For this review, take the finished solid that the model builds, in its own axes (mm). Face numbers are marked on the shaded views. A direction names the side the tool comes from. Give positions to 0.01 mm unless a question says otherwise; leave off trailing zeros. Write each loop counter-clockwise with the first axis right and the second up, starting at its lowest first coordinate (ties: lowest second). Pieces come first, ordered by that corner, then holes.
1) Machinability: for the marked faces 5, 6, 7 and 8, which of the approach directions +Z, -Z, +X, -X, +Y, -Y give a long, thin tool a straight path to every point of the face, cutting with its end or side? Answer none if there is none.
2) Draft analysis for pull direction Y (two halves, no side actions). For the marked faces 1, 2, 3 and 4, state which applies: pulls with the +Y half, pulls with the -Y half, needs draft (parallel to the pull), parting line crosses it, or undercut.
3) We need section C-C on z = -5. Give the boundary of the cut face in (x, y).
4) For P1, Ø3, axis at x = 12.5, z = 9.5, coming from the -Y side; P2, Ø2, axis at x = 26.5, y = -0.5, coming from the -Z side; P3, Ø2.5, axis at y = 6, z = 8.5, coming from the -X side; P4, Ø8.5, axis at x = 0, y = 0, coming from the +Z side, all flat-tipped, find the tip position at first contact; note any pin that passes through.
5) We need section B-B on z = 10. Give the boundary of the cut face in (x, y), and give its area (3 significant figures).
6) Wall thickness on line 1 along Y through (x, z) = (0, -7.25); line 2 along Z through (x, y) = (-16, -20); line 3 along Z through (x, y) = (18.5, -28.5): over which ranges is each line inside the solid? List them lowest first.
7) We need section A-A on x = 0. Give the boundary of the cut face in (y, z).
8) We need section D-D on y = -15. Give the boundary of the cut face in (x, z), and give its area (3 significant figures).
from build123d import *

# Parameters (mm, degrees)
BACK_DISC_SKETCH_R        = 37.5
BACK_DISC_75_DEPTH        = 3
BLADES_6X_DEPTH           = 14
HUB_SKETCH_R              = 12.5
HUB_25_DEPTH              = 16
KEYED_SHAFT_BORE_14_DEPTH = 63.461988441


with BuildPart() as part:
    # Back Disc Sketch → Back Disc Ø75 (new body)
    with BuildSketch(Plane.XY):
        Circle(BACK_DISC_SKETCH_R)
    extrude(amount=BACK_DISC_75_DEPTH)

    # Blade Profiles Sketch → Blades 6x (add)
    with BuildSketch(Plane.XY.offset(3)):
        with BuildLine():
            ThreePointArc((3.63084944, 16.288815705), (11.178007051, 25.36087614), (21.79252918, 30.51779271))
            Line((21.79252918, 30.51779271), (18.431665522, 32.657674536))
            ThreePointArc((18.431665522, 32.657674536), (8.308835539, 26.888544841), (1.030700016, 17.790012675))
            Line((1.030700016, 17.790012675), (3.63084944, 16.288815705))
        make_face()
        with BuildLine():
            ThreePointArc((-12.291103478, 11.288815705), (-16.374159474, 22.36087614), (-15.532919164, 34.131780238))
            Line((-15.532919164, 34.131780238), (-19.066543016, 32.291127844))
            ThreePointArc((-19.066543016, 32.291127844), (-19.131745134, 20.639935074), (-14.891252903, 9.787618735))
            Line((-14.891252903, 9.787618735), (-12.291103478, 11.288815705))
        make_face()
        with BuildLine():
            ThreePointArc((-15.921952918, -5), (-27.552166525, -3), (-37.325448345, 3.613987528))
            Line((-37.325448345, 3.613987528), (-37.498208538, -0.366546692))
            ThreePointArc((-37.498208538, -0.366546692), (-27.440580673, -6.248609768), (-15.921952918, -8.00239394))
            Line((-15.921952918, -8.00239394), (-15.921952918, -5))
        make_face()
        with BuildLine():
            ThreePointArc((-3.63084944, -16.288815705), (-11.178007051, -25.36087614), (-21.79252918, -30.51779271))
            Line((-21.79252918, -30.51779271), (-18.431665522, -32.657674536))
            ThreePointArc((-18.431665522, -32.657674536), (-8.308835539, -26.888544841), (-1.030700016, -17.790012675))
            Line((-1.030700016, -17.790012675), (-3.63084944, -16.288815705))
        make_face()
        with BuildLine():
            ThreePointArc((12.291103478, -11.288815705), (16.374159474, -22.36087614), (15.532919164, -34.131780238))
            Line((15.532919164, -34.131780238), (19.066543016, -32.291127844))
            ThreePointArc((19.066543016, -32.291127844), (19.131745134, -20.639935074), (14.891252903, -9.787618735))
            Line((14.891252903, -9.787618735), (12.291103478, -11.288815705))
        make_face()
        with BuildLine():
            ThreePointArc((15.921952918, 5), (27.552166525, 3), (37.325448345, -3.613987528))
            Line((37.325448345, -3.613987528), (37.498208538, 0.366546692))
            ThreePointArc((37.498208538, 0.366546692), (27.440580673, 6.248609768), (15.921952918, 8.00239394))
            Line((15.921952918, 8.00239394), (15.921952918, 5))
        make_face()
    extrude(amount=BLADES_6X_DEPTH)

    # Hub Sketch → Hub Ø25 (add)
    with BuildSketch(Plane(origin=(0, 0, 0), x_dir=(-1, 0, 0), z_dir=(0, 0, -1))):
        Circle(HUB_SKETCH_R)
    extrude(amount=HUB_25_DEPTH)

    # Shaft Bore Sketch → Keyed Shaft Bore Ø14 (cut, through all)
    with BuildSketch(Plane(origin=(0, 0, -16), x_dir=(-1, 0, 0), z_dir=(0, 0, -1))):
        with BuildLine():
            Line((-2.5, 6.538348415), (-2.5, 9.3))
            Line((-2.5, 9.3), (2.5, 9.3))
            Line((2.5, 9.3), (2.5, 6.538348415))
            ThreePointArc((2.5, 6.538348415), (0, -7), (-2.5, 6.538348415))
        make_face()
    extrude(amount=-KEYED_SHAFT_BORE_14_DEPTH, mode=Mode.SUBTRACT)


solid = part.part
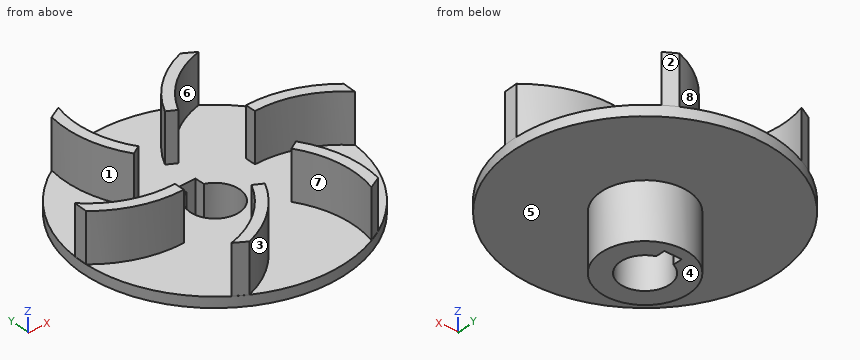
Results list:
1. face 5: -Z
1. face 6: +Z, +X
1. face 7: +Z
1. face 8: +Z, +Y
2. face 1: undercut
2. face 2: pulls with the +Y half
2. face 3: pulls with the -Y half
2. face 4: needs draft
3. outline: circle Ø25 at (0, 0); hole (-2.5, 6.54) arc R7 ccw (long way) to (2.5, 6.54) - (2.5, 9.3) - (-2.5, 9.3) - close
4. P1: stops at y = -14.4
4. P2: stops at z = 0
4. P3: stops at x = 15.92
4. P4: passes through
5. outline: (-37.5, -0.37) arc R31 ccw to (-15.92, -8) - (-15.92, -5) arc R28 cw to (-37.33, 3.61) - close; (-21.79, -30.52) - (-18.43, -32.66) arc R31 ccw to (-1.03, -17.79) - (-3.63, -16.29) arc R28 cw to start; (-19.07, 32.29) arc R31 ccw to (-14.89, 9.79) - (-12.29, 11.29) arc R28 cw to (-15.53, 34.13) - close; (1.03, 17.79) - (3.63, 16.29) arc R28 cw to (21.79, 30.52) - (18.43, 32.66) arc R31 ccw to start; (12.29, -11.29) arc R28 cw to (15.53, -34.13) - (19.07, -32.29) arc R31 ccw to (14.89, -9.79) - close; (15.92, 5) arc R28 cw to (37.33, -3.61) - (37.5, 0.37) arc R31 ccw to (15.92, 8) - close
5. area: 425 mm2
6. line 1: y = -12.5 to -7, 9.3 to 12.5
6. line 2: z = 0 to 3
6. line 3: z = 0 to 17
7. outline: (-37.5, 0) - (-12.5, 0) - (-12.5, -16) - (-7, -16) - (-7, 3) - (-37.5, 3) - close; (9.3, -16) - (12.5, -16) - (12.5, 0) - (37.5, 0) - (37.5, 3) - (9.3, 3) - close
8. outline: (-34.37, 0) - (34.37, 0) - (34.37, 3) - (17.52, 3) - (17.52, 17) - (14.27, 17) - (14.27, 3) - (-34.37, 3) - close
8. area: 252 mm2
